from build123d import *

# Parameters (mm, degrees)
SKETCH1_R          = 18.4
BASE_EXTRUDE_DEPTH = 32.54375
SKETCH2_OUTSIDE_W  = 485.848
SKETCH2_OUTSIDE_H  = 494.398
SKETCH2_OUTSIDE_R  = 28.1
CUT_EXTRUDE1_DEPTH = 54.833293767
CUT_EXTRUDE1_DRAFT = -75
SKETCH3_OUTSIDE_W  = 485.848
SKETCH3_OUTSIDE_H  = 494.398
SKETCH3_OUTSIDE_R  = 28.1
CUT_EXTRUDE2_DEPTH = 54.833293767
CUT_EXTRUDE2_DRAFT = -75
CHAMFER1_SIZE      = 2.307142857


with BuildPart() as part:
    # Sketch1 → Base-Extrude (new body)
    with BuildSketch(Plane.XY):
        Polygon((0.127390736, 32.384749445), (-27.982320346, 16.302698336), (-28.109711083, -16.082051108), (-0.127390736, -32.384749445), (27.982320346, -16.302698336), (28.109711083, 16.082051108), align=None)
        Circle(SKETCH1_R, mode=Mode.SUBTRACT)
    extrude(amount=BASE_EXTRUDE_DEPTH)


with BuildPart() as cut_extrude1_tool:
    # Sketch2 outside → Cut-Extrude1 (with draft: the straight prism first)
    with BuildSketch(Plane(origin=(0, 0, 0), x_dir=(-1, 0, 0), z_dir=(0, 0, -1))):
        Rectangle(SKETCH2_OUTSIDE_W, SKETCH2_OUTSIDE_H)
        Circle(SKETCH2_OUTSIDE_R, mode=Mode.SUBTRACT)
    extrude(amount=-CUT_EXTRUDE1_DEPTH)
    # Cut-Extrude1: the draft: its side faces are tilted about the plane it starts from
    cut_extrude1_sides = [cut_extrude1_tool.faces().sort_by_distance(p)[0] for p in [
        (0, -247.199, 27.416646884),
        (-242.924, 0, 27.416646884),
        (0, 247.199, 27.416646884),
        (242.924, 0, 27.416646884),
        (28.1, 0, 27.416646884),
    ]]
    draft(cut_extrude1_sides, Plane(origin=(0, 0, 0), x_dir=(-1, 0, 0), z_dir=(0, 0, -1)), CUT_EXTRUDE1_DRAFT)


with BuildPart() as part_1:
    add(part.part)

    # Cut-Extrude1: cut by cut_extrude1_tool
    add(cut_extrude1_tool.part, mode=Mode.SUBTRACT)


with BuildPart() as cut_extrude2_tool:
    # Sketch3 outside → Cut-Extrude2 (with draft: the straight prism first)
    with BuildSketch(Plane.XY.offset(32.54375)):
        Rectangle(SKETCH3_OUTSIDE_W, SKETCH3_OUTSIDE_H)
        Circle(SKETCH3_OUTSIDE_R, mode=Mode.SUBTRACT)
    extrude(amount=-CUT_EXTRUDE2_DEPTH)
    # Cut-Extrude2: the draft: its side faces are tilted about the plane it starts from
    cut_extrude2_sides = [cut_extrude2_tool.faces().sort_by_distance(p)[0] for p in [
        (0, -247.199, 5.127103116),
        (242.924, 0, 5.127103116),
        (0, 247.199, 5.127103116),
        (-242.924, 0, 5.127103116),
        (-28.1, 0, 5.127103116),
    ]]
    draft(cut_extrude2_sides, Plane.XY.offset(32.54375), CUT_EXTRUDE2_DRAFT)


with BuildPart() as part_2:
    add(part_1.part)

    # Cut-Extrude2: cut by cut_extrude2_tool
    add(cut_extrude2_tool.part, mode=Mode.SUBTRACT)

    # Chamfer1
    chamfer1_edges = [part_2.edges().sort_by_distance(p)[0] for p in [
        (-18.4, 0, 0),
        (-18.4, 0, 32.54375),
    ]]
    chamfer(chamfer1_edges, length=CHAMFER1_SIZE)


solid = part_2.part
For this review, take the finished solid that the model builds, in its own axes (mm). Coordinates: 2 decimals unless noted, no trailing zeros. Order: outer loops, then holes, each group sorted by start corner. A loop starts at its lowest first (then second) coordinate and runs counter-clockwise, first axis right, second up. Notation, with made-up numbers: (12, 33) - (34, 33) arc R20 cw to (34, 38) - close; hole circle Ø1 at (58, -28.5). An arc over 180 degrees is marked (long way). Answer as CSV lines item,"result". Start each with the question number.
1) Insertion check: P1, Ø1, axis at y = -4.5, z = 23, coming from the -X side; P2, Ø6, axis at x = -15, z = 15.5, coming from the -Y side; P3, Ø8, axis at x = -1, z = 21.5, coming from the +Y side. Each pin has a flat end and moves straight along its axis. Give the tip position at first contact, or say it passes through.
2) To check wall thickness, follow line 1 along Y through (x, z) = (0, 9); line 2 along Y through (x, z) = (8.5, 20.5); line 3 along X through (y, z) = (9.5, 27). State the ranges of each line that lie inside material, in increasing order. Write a range as [from, to].
3) Draft analysis for pull direction X (two halves, no side actions). For faces 1 (the conical face through (-2.41, 18.354, 30.349)), 2 (the conical face through (0.18, 29.12, 32.27)), 3 (the conical face through (-25.246, -14.516, 0.274)), state which applies: +X half, -X half, draft (parallel to the pull), parting line (faces both ways), or undercut.
4) Add section A-A (z = 7.5). State the section outline as (x, y) points.
5) Add section B-B (y = 0). State the section outline as (x, z) points, then the cut area to 3 significant figures.
Result:
1,P1,"x = -28.07"
1,P2,"y = -25.47"
1,P3,"y = 32.38"
2,line 1,"[-32.31, -18.4], [18.4, 32.31]"
2,line 2,"[-27.45, -16.32], [16.32, 27.51]"
2,line 3,"[-28.01, -15.76], [15.76, 28.08]"
3,face 1,"undercut"
3,face 2,"parting line"
3,face 3,"-X half"
4,outline,"(-28.11, -16.08) - (-0.13, -32.38) - (27.98, -16.3) - (28.11, 16.08) - (0.13, 32.38) - (-27.98, 16.3) - close; hole circle Ø36.8 at (0, 0)"
5,outline,"(-28.05, 0) - (-20.71, 0) - (-18.4, 2.31) - (-18.4, 30.24) - (-20.71, 32.54) - (-28.05, 32.54) - close; (18.4, 2.31) - (20.71, 0) - (28.05, 0) - (28.05, 32.54) - (20.71, 32.54) - (18.4, 30.24) - close"
5,area,"617 mm^2"
